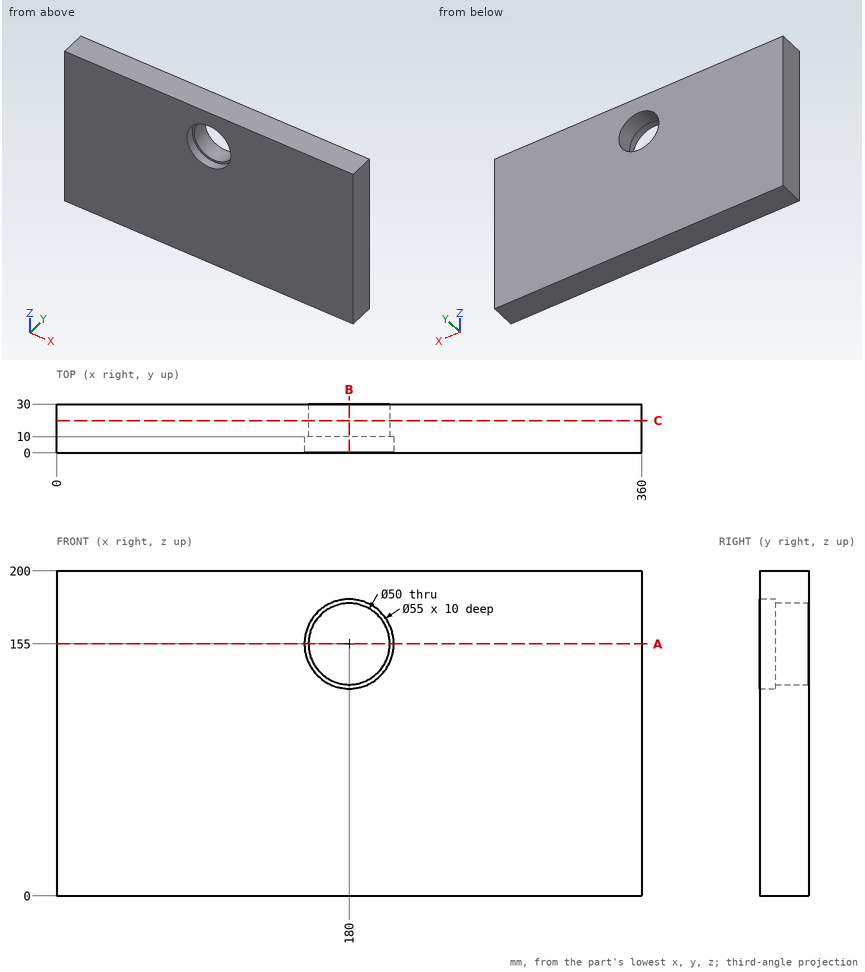
Could you check a few things on this drawing? It's one solid part, dimensions in mm from its lowest x, y, z. Round coordinates to 2 decimals unless told otherwise and drop trailing zeros. Order: outer loops, then holes, each group sorted by start corner. A loop starts at its lowest first (then second) coordinate and runs counter-clockwise, first axis right, second up. Notation, with made-up numbers: M 42,28 L 71,28 A25 cw 71,52 Z; hole C 61,43.25 d1. An arc over 180 degrees is marked long. Return JSON: item names as keys, results as strings. Group by question number.
1. I'm going to push a flat-ended pin straight in: pin 1 Ø6 at (x, y) = (323, 4.5) entering from -Z. Where does the tip first touch, or does it pass through?
2. Please list where these lines run through material, in increasing order: probe 1 along X at (y, z) = (6.25, 155); probe 2 along X at (y, z) = (2.5, 157); probe 3 along Z at (x, y) = (174, 3.75).
3. If we section it at C-C on y = 19.75: List the corners of the cut face in (x, z) for me, then the cut area to 3 significant figures.
4. If we section it at A-A on z = 155: List the corners of the cut face in (x, y) for me.
5. If we section it at B-B on x = 180: List the corners of the cut face in (y, z) for me.
Reply:
{
 "1": {"pin 1": "z = 0"},
 "2": {"probe 1": "0 to 152.5, 207.5 to 360", "probe 2": "0 to 152.57, 207.43 to 360", "probe 3": "0 to 128.16, 181.84 to 200"},
 "3": {"outline": "M 0,0 L 360,0 L 360,200 L 0,200 Z; hole C 180,155 d50", "area": "70,000 mm^2"},
 "4": {"outline": "M 0,0 L 152.5,0 L 152.5,10 L 155,10 L 155,30 L 0,30 Z; M 205,10 L 207.5,10 L 207.5,0 L 360,0 L 360,30 L 205,30 Z"},
 "5": {"outline": "M 0,0 L 30,0 L 30,130 L 10,130 L 10,127.5 L 0,127.5 Z; M 0,182.5 L 10,182.5 L 10,180 L 30,180 L 30,200 L 0,200 Z"}
}
